Read the model definition and answer for the solid it produces. Units are mm, in the model's axes. A direction names the side the tool comes from. Give positions to 0.01 mm unless a question says otherwise; leave off trailing zeros. Write each loop counter-clockwise with the first axis right and the second up, starting at its lowest first coordinate (ties: lowest second). Pieces come first, ordered by that corner, then holes.
```python
from build123d import *

# Parameters (mm, degrees)
BOSS_EXTRUDE1_DEPTH = 12
FILLET1_R           = 3
FILLET2_R           = 3
SKETCH2_R           = 1.5
CUT_EXTRUDE1_DEPTH  = 33.32645975
SKETCH3_R           = 4
BOSS_EXTRUDE2_DEPTH = 116
SKETCH4_R           = 6.081663029
BOSS_EXTRUDE3_DEPTH = 3


with BuildPart() as part:
    # Sketch1 → Boss-Extrude1 (new body)
    with BuildSketch(Plane.XY):
        Polygon((0, 26), (0, 0), (15, 0), (15, 26), (12, 26), (12, 3), (3, 3), (3, 26), align=None)
    extrude(amount=BOSS_EXTRUDE1_DEPTH)

    # Fillet1
    fillet1_edges = [part.edges().sort_by_distance(p)[0] for p in [
        (1.5, 26, 0),
        (13.5, 26, 12),
        (1.5, 26, 12),
        (13.5, 26, 0),
    ]]
    fillet(fillet1_edges, radius=FILLET1_R)

    # Fillet2
    fillet2_edges = [part.edges().sort_by_distance(p)[0] for p in [
        (3, 3, 6),
        (12, 3, 6),
    ]]
    fillet(fillet2_edges, radius=FILLET2_R)

    # Sketch2 → Cut-Extrude1 (cut, through all)
    with BuildSketch(Plane(origin=(15, 0, 0), x_dir=(0, 0, -1), z_dir=(1, 0, 0))):
        with Locations(Location((-6, 20, 0), (0, 0, 90))):
            Circle(SKETCH2_R)
    extrude(amount=-CUT_EXTRUDE1_DEPTH, mode=Mode.SUBTRACT)

    # Sketch3 → Boss-Extrude2 (add)
    with BuildSketch(Plane(origin=(0, 0, 0), x_dir=(-1, 0, 0), z_dir=(0, -1, 0))):
        with Locations(Location((-7.5, -6, 0), (0, 0, 270))):
            Circle(SKETCH3_R)
    extrude(amount=BOSS_EXTRUDE2_DEPTH)

    # Sketch4 → Boss-Extrude3 (add)
    with BuildSketch(Plane(origin=(0, -116, 0), x_dir=(-1, 0, 0), z_dir=(0, -1, 0))):
        with Locations(Location((-7.5, -6, 0), (0, 0, 90))):
            Circle(SKETCH4_R)
    extrude(amount=BOSS_EXTRUDE3_DEPTH)


solid = part.part
```
Item 1: Which of the six approach directions +Z, -Z, +X, -X, +Y, -Y give full straight-line access (tool end or side, diameter ignored) to faces 1 (the cylindrical face through (11.1, 3.86, 6.08)), 2 (the cylindrical face through (1.563, -117.479, 7.318)), 3 (the flat face through (4, 0, 3))?
Result set:
face 1: +Z, -Z, +Y
face 2: -Y
face 3: none
Item 2: Section A-A (y = 20) is taken. Write down the section's boundary in (x, z), and give its area (3 significant figures).
Result set:
outline: (0, 0) - (3, 0) - (3, 4.5) - (0, 4.5) - close; (0, 7.5) - (3, 7.5) - (3, 12) - (0, 12) - close; (12, 0) - (15, 0) - (15, 4.5) - (12, 4.5) - close; (12, 7.5) - (15, 7.5) - (15, 12) - (12, 12) - close
area: 54.0 mm2
Item 3: Each of these flat-tipped pins is pushed along its axis until it touches: pin 1 Ø3.5 at (x, z) = (9.5, 5) entering from +Y; pin 2 Ø7.5 at (x, y) = (8, 6) entering from +Z; pin 3 Ø6 at (y, z) = (-6.5, 2.5) entering from +X. Where does it stop, or does it pass through?
Result set:
pin 1: stops at y = 4.02
pin 2: stops at z = 12
pin 3: stops at x = 11.47
Item 4: Section C-C (x = 7.5) is taken. Write down the section's boundary in (y, z).
Result set:
outline: (-119, -0.08) - (-116, -0.08) - (-116, 2) - (0, 2) - (0, 0) - (3, 0) - (3, 12) - (0, 12) - (0, 10) - (-116, 10) - (-116, 12.08) - (-119, 12.08) - close
Item 5: Section D-D (y = -11) is taken. Write down the section's boundary in (x, z).
Result set:
outline: circle Ø8 at (7.5, 6)
Item 6: Section B-B (z = 6) is taken. Write down the section's boundary in (x, y), and give its area (3 significant figures).
Result set:
outline: (0, 0) - (3.5, 0) - (3.5, -116) - (1.42, -116) - (1.42, -119) - (13.58, -119) - (13.58, -116) - (11.5, -116) - (11.5, 0) - (15, 0) - (15, 18.5) - (12, 18.5) - (12, 6) arc R3 cw to (9, 3) - (6, 3) arc R3 cw to (3, 6) - (3, 18.5) - (0, 18.5) - close; (0, 21.5) - (3, 21.5) - (3, 26) - (0, 26) - close; (12, 21.5) - (15, 21.5) - (15, 26) - (12, 26) - close
area: 1,130 mm2
Item 7: Determine the mould class of faces 4 (the cylindrical face through (13.52, 18.5, 6.07)), 5 (the cylindrical face through (6.299, -57.188, 9.815)), 6 (the cylindrical face through (1.48, 25.14, 11.1)) for opening direction Z: pulls with the +Z half, pulls with the -Z half, needs draft (parallel to the pull), parting line crosses it, or undercut.
Result set:
face 4: undercut
face 5: parting line crosses it
face 6: pulls with the +Z half
Item 8: Find the intervals of material crossed by line 1 along Z through (x, y) = (0.9, 20); line 2 along Y through (x, z) = (7.75, 10.5); line 3 along Y through (x, z) = (13, 5.5), in increasing order.
Result set:
line 1: z = 0 to 4.5, 7.5 to 12
line 2: y = -119 to -116, 0 to 3
line 3: y = -119 to -116, 0 to 18.59, 21.41 to 26
